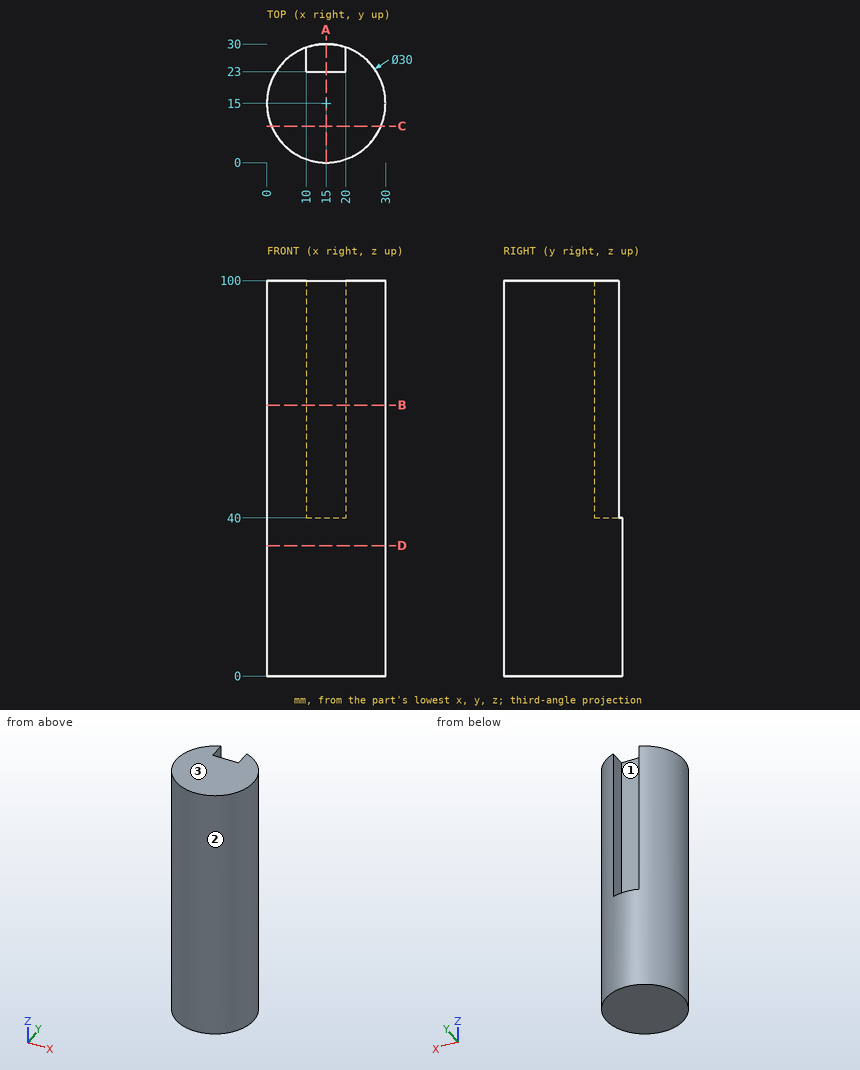
Check sheet for the drawn part. Datum: minimum x, y, z corner. Units: mm. Give positions to 0.01 mm unless a question says otherwise; leave off trailing zeros. Write each loop counter-clockwise with the first axis right and the second up, starting at its lowest first coordinate (ties: lowest second). Pieces come first, ordered by that corner, then holes. Notation, with made-up numbers: (25.5, 34) -> (73.5, 34) arc R23 ccw to (73.5, 63) -> close; hole circle Ø4 at (54.5, 86). An arc over 180 degrees is marked (long way). Use one line per item in the form item = value. Start each with the question number.
1. Thickness scan on line 1 along Z through (x, y) = (18, 24.5); line 2 along X through (y, z) = (14.25, 63.5); line 3 along Y through (x, z) = (15.75, 76.5). Record the ranges inside material, lowest first. Write a range as from..to.
2. Go/stop test with flat-tipped pins: P1, Ø5, axis at y = 27, z = 23, coming from the -X side; P2, Ø1.5, axis at x = 21.5, z = 26, coming from the +Y side; P3, Ø2, axis at x = 17, z = 53, coming from the +Y side. Record where each tip stops, or that it passes through.
3. Section check C-C (y = 9.25). Record the cut outline in (x, z), and give its area (3 significant figures).
4. Section check A-A (x = 15). Record the cut outline in (y, z).
5. Section check D-D (z = 33). Record the cut outline in (x, y).
6. Section check B-B (z = 68.5). Record the cut outline in (x, y).
7. Mould release check, pull along X, two halves, no side actions. Record for the marked faces 1, 2 and 3: pulls with the +X half, pulls with the -X half, needs draft (parallel to the pull), parting line crosses it, or undercut.
Conclusion:
q1.line_1 = 0..40
q1.line_2 = 0.02..29.98
q1.line_3 = 0.02..23
q2.P1 = 3.39
q2.P2 = 28.85
q2.P3 = 23
q3.outline = (1.15, 0) -> (28.85, 0) -> (28.85, 100) -> (1.15, 100) -> close
q3.area = 2,770 mm²
q4.outline = (0, 0) -> (30, 0) -> (30, 40) -> (23, 40) -> (23, 100) -> (0, 100) -> close
q5.outline = circle Ø30 at (15, 15)
q6.outline = (10, 23) -> (10, 29.14) arc R15 ccw (long way) to (20, 29.14) -> (20, 23) -> close
q7.face_1 = undercut
q7.face_2 = parting line crosses it
q7.face_3 = needs draft
